For this review, take the finished solid that the model builds, in its own axes (mm). Face numbers are marked on the shaded views. A direction names the side the tool comes from. Coordinates: 2 decimals unless noted, no trailing zeros. Loops run counter-clockwise (first coordinate to the right, second up) from the corner with the lowest first, then second, coordinate; pieces in that order, holes last.
1. Clearance check with flat-ended pins moving along their axes: P1, Ø8, axis at x = -38.97, y = -22.5, coming from the +Z side; P2, Ø16, axis at x = 0, z = 34, coming from the -Y side; P3, Ø12, axis at x = 38.5, y = 40, coming from the -Z side; P4, Ø1, axis at y = -9, z = 39.5, coming from the -X side. State where each tip first meets the part, or that it passes through.
2. Machinability: for the marked faces 4 and 5, which of the approach directions +Z, -Z, +X, -X, +Y, -Y give a long, thin tool a straight path to every point of the face, cutting with its end or side? Answer none if there is none.
3. Take a section at D-D, the plane y = -45. State the section outline as (x, z) points, then the cut area to 3 significant figures.
4. Take a section at C-C, the plane y = 22.5. State the section outline as (x, z) points.
5. Take a section at A-A, the plane x = 0. State the section outline as (y, z) points, then the cut area to 3 significant figures.
6. To check wall thickness, follow probe 1 along Z at (x, y) = (0, -17); probe 2 along Z at (x, y) = (-29, -35.5); probe 3 along X at (y, z) = (4, 20). State the ranges of each line that lie inside material, in increasing order.
7. Take a section at B-B, the plane z = 4.5. State the section outline as (x, y) points.
8. Mouldability with a two-part tool opening along X and no side actions: class the marked faces 1, 2 and 3 as pulls with the +X half, pulls with the -X half, needs draft (parallel to the pull), parting line crosses it, or undercut.
```python
from build123d import *

# Parameters (mm, degrees)
SKETCH1_R               = 52.5
SKETCH1_R_2             = 3.5
BOSS_EXTRUDE1_DEPTH     = 14
SKETCH2_R               = 25
SKETCH2_R_2             = 10
BOSS_EXTRUDE2_DEPTH     = 35
CUT_EXTRUDE1_DEPTH      = 89.95785519
CUT_EXTRUDE1_DEPTH_BACK = 89.95785519
SKETCH3_R               = 5


with BuildPart() as part:
    # Sketch1 → Boss-Extrude1 (new body)
    with BuildSketch(Plane.XY):
        Circle(SKETCH1_R)
        with Locations((0, 45)):
            Circle(SKETCH1_R_2, mode=Mode.SUBTRACT)
        with Locations((38.97114317, 22.5)):
            Circle(SKETCH1_R_2, mode=Mode.SUBTRACT)
        with Locations((38.97114317, -22.5)):
            Circle(SKETCH1_R_2, mode=Mode.SUBTRACT)
        with Locations((0, -45)):
            Circle(SKETCH1_R_2, mode=Mode.SUBTRACT)
        with Locations((-38.97114317, -22.5)):
            Circle(SKETCH1_R_2, mode=Mode.SUBTRACT)
        with Locations((-38.97114317, 22.5)):
            Circle(SKETCH1_R_2, mode=Mode.SUBTRACT)
    extrude(amount=BOSS_EXTRUDE1_DEPTH)

    # Sketch2 → Boss-Extrude2 (add)
    with BuildSketch(Plane.XY.offset(14)):
        Circle(SKETCH2_R)
        Circle(SKETCH2_R_2, mode=Mode.SUBTRACT)
    extrude(amount=BOSS_EXTRUDE2_DEPTH)

    # Sketch3 → Cut-Extrude1 (cut, two sides: drawn at the far end of the back side and taken through both)
    with BuildSketch(Plane(origin=(0, 0, 0), x_dir=(1, 0, 0), z_dir=(0, 1, 0)).offset(-CUT_EXTRUDE1_DEPTH_BACK)):
        with Locations(Location((0, -34, 0), (0, 0, 270))):
            Circle(SKETCH3_R)
    extrude(amount=CUT_EXTRUDE1_DEPTH + CUT_EXTRUDE1_DEPTH_BACK, mode=Mode.SUBTRACT)


solid = part.part
```
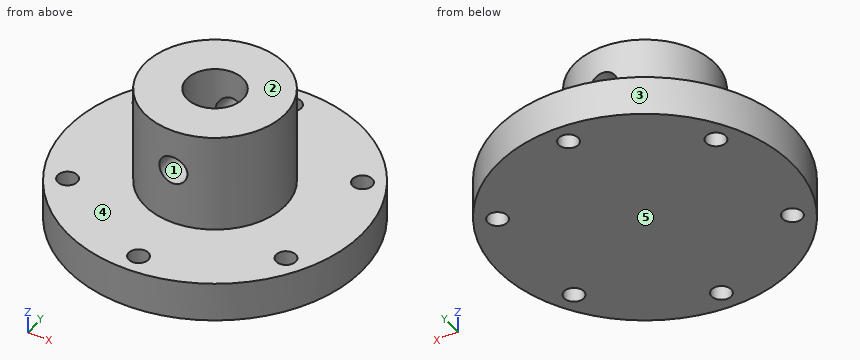
Results list:
1. P1: stops at z = 14
1. P2: stops at y = -25
1. P3: stops at z = 0
1. P4: stops at x = -23.51
2. face 4: +Z
2. face 5: -Z, +X, -X, +Y, -Y
3. outline: (-27.04, 0) - (-3.5, 0) - (-3.5, 14) - (-27.04, 14) - close; (3.5, 0) - (27.04, 0) - (27.04, 14) - (3.5, 14) - close
3. area: 659 mm2
4. outline: (-47.43, 0) - (-42.47, 0) - (-42.47, 14) - (-47.43, 14) - close; (-35.47, 0) - (35.47, 0) - (35.47, 14) - (10.9, 14) - (10.9, 49) - (-10.9, 49) - (-10.9, 14) - (-35.47, 14) - close; (42.47, 0) - (47.43, 0) - (47.43, 14) - (42.47, 14) - close; hole circle Ø10 at (0, 34)
5. outline: (-52.5, 0) - (-48.5, 0) - (-48.5, 14) - (-52.5, 14) - close; (-41.5, 0) - (41.5, 0) - (41.5, 14) - (25, 14) - (25, 29) - (10, 29) - (10, 14) - (-10, 14) - (-10, 29) - (-25, 29) - (-25, 14) - (-41.5, 14) - close; (-25, 39) - (-10, 39) - (-10, 49) - (-25, 49) - close; (10, 39) - (25, 39) - (25, 49) - (10, 49) - close; (48.5, 0) - (52.5, 0) - (52.5, 14) - (48.5, 14) - close
5. area: 2,020 mm2
6. probe 1: z = 0 to 29, 39 to 49
6. probe 2: z = 0 to 14
6. probe 3: x = -24.68 to -9.17, 9.17 to 24.68
7. outline: circle Ø105 at (0, 0); hole circle Ø7 at (-38.97, -22.5); hole circle Ø7 at (-38.97, 22.5); hole circle Ø7 at (0, -45); hole circle Ø7 at (0, 45); hole circle Ø7 at (38.97, -22.5); hole circle Ø7 at (38.97, 22.5)
8. face 1: undercut
8. face 2: needs draft
8. face 3: parting line crosses it
